For this review, take the finished solid that the model builds, in its own axes (mm). Coordinates: 2 decimals unless noted, no trailing zeros. Order: outer loops, then holes, each group sorted by start corner. A loop starts at its lowest first (then second) coordinate and runs counter-clockwise, first axis right, second up. Notation, with made-up numbers: (-18.75, 86.5) -> (-5.75, 86.5) arc R36 ccw to (-5.75, 125.5) -> close; hole circle Ø2 at (2, -31.5). An arc over 180 degrees is marked (long way). Write item = value, one per line. Start each with the question number.
1) Consider section A-A on z = 0. Give the boundary of the cut face in (x, y), and give its area (3 significant figures).
2) Consider section C-C on y = 760.5. Give the boundary of the cut face in (x, z).
3) Insertion check: pin 1 Ø2 at (y, z) = (577.5, -2) entering from -X; pin 2 Ø2 at (y, z) = (541, 0) entering from +X; pin 3 Ø1.5 at (x, z) = (303.5, 2) entering from +Y. Each pin has a flat end and moves straight along its axis. Give the tip position at first contact, or say it passes through.
4) Consider section B-B on x = 516.5. Give the boundary of the cut face in (y, z), and give its area (3 significant figures).
5) Wall thickness on probe 1 along Y at (x, z) = (276, 0); probe 2 along X at (y, z) = (619.5, 0.75); probe 3 along X at (y, z) = (685, 1.25): over which ranges is each line inside the solid? List them lowest first. Write a range as [from, to].
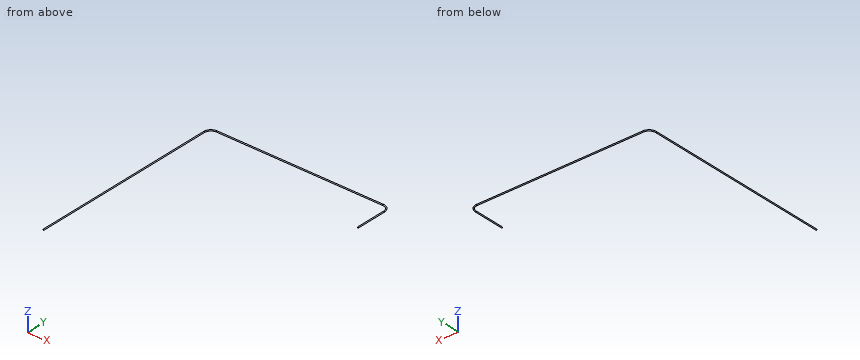
from build123d import *

# Parameters (mm, degrees)
SKETCH2_R = 3.25


with BuildPart() as part:
    # Sweep1: sweep along a path in Sketch1
    with BuildLine(Plane.XY) as sweep1_path:
        Line((0, 0), (0, 1153))
        ThreePointArc((0, 1153), (12.30151519, 1182.69848481), (42, 1195))
        Line((42, 1195), (1060, 1195))
        ThreePointArc((1060, 1195), (1089.69848481, 1182.69848481), (1102, 1153))
        Line((1102, 1153), (1102, 965))
    # Sketch2 → Sweep1 (sweep)
    with BuildSketch(Plane(origin=(0, 0, 0), x_dir=(1, 0, 0), z_dir=(0, 1, 0))):
        Circle(SKETCH2_R)
    sweep(path=sweep1_path.line)


solid = part.part
Answer sheet:
q1.outline = (-3.25, 0) -> (3.25, 0) -> (3.25, 1153) arc R38.75 cw to (42, 1191.75) -> (1060, 1191.75) arc R38.75 cw to (1098.75, 1153) -> (1098.75, 965) -> (1105.25, 965) -> (1105.25, 1153) arc R45.25 ccw to (1060, 1198.25) -> (42, 1198.25) arc R45.25 ccw to (-3.25, 1153) -> close
q1.area = 16,200 mm2
q2.outline = circle Ø6.5 at (0, 0)
q3.pin_1 = -3.09
q3.pin_2 = 3.25
q3.pin_3 = 1198
q4.outline = circle Ø6.5 at (1195, 0)
q4.area = 33.2 mm2
q5.probe_1 = [1191.75, 1198.25]
q5.probe_2 = [-3.16, 3.16]
q5.probe_3 = [-3, 3]
